Part print with two shaded views. Sizes in mm from the minimum x, y, z corner. A direction names the side the tool comes from. Round coordinates to 2 decimals unless told otherwise and drop trailing zeros. Order: outer loops, then holes, each group sorted by start corner. A loop starts at its lowest first (then second) coordinate and runs counter-clockwise, first axis right, second up. Notation, with made-up numbers: M 41,78 L 69,78 A8 cw 69,93 Z; hole C -34,54.5 d3. An arc over 180 degrees is marked long. Answer as a JSON object with one key per item and string values.
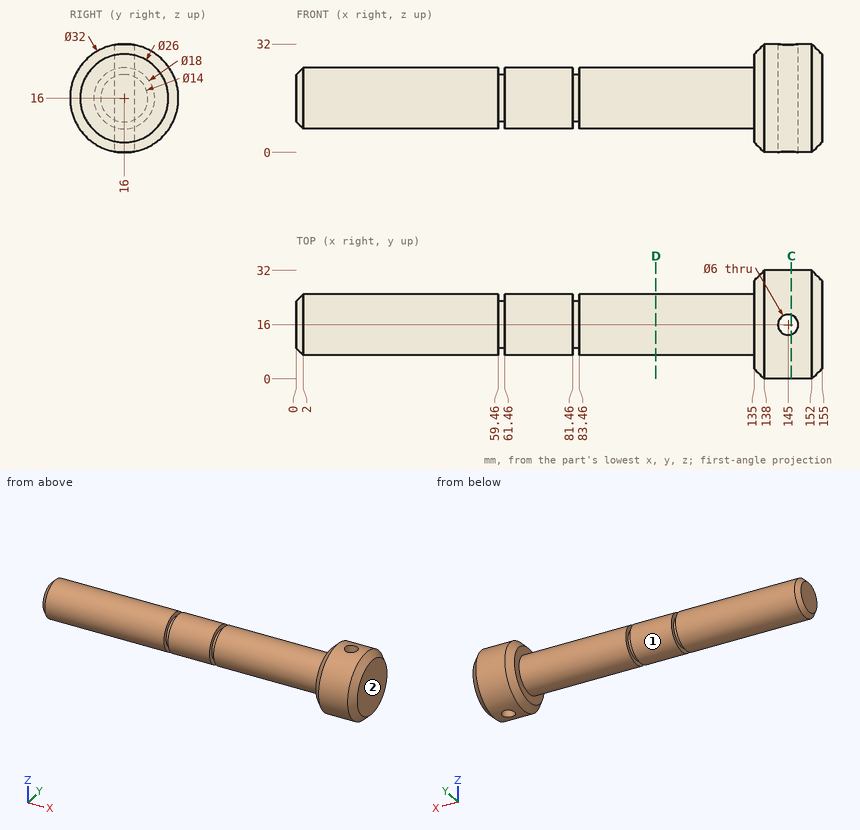
Item 1: Wall check: line 1 along Y through (x, z) = (145, 14); line 2 along X through (y, z) = (23.5, 9.5); line 3 along Y through (x, z) = (145, 7). Give the ranges that are in metal, low to high. Write a range as [from, to].
Worked answers:
{"line 1": "y = [0.13, 13], [19, 31.87]", "line 2": "x = [135, 155]", "line 3": "y = [2.77, 13], [19, 29.23]"}
Item 2: 3-axis set-ups, long thin cutter, end or side, ignore diameter. For the marked faces 1 and 2: which of +Z, -Z, +X, -X, +Y, -Y reach the whole face in a straight line?
Worked answers:
{"face 1": "-X", "face 2": "+Z, -Z, +X, +Y, -Y"}
Item 3: Drop flat-ended pins along their axis: pin 1 Ø12 at (x, z) = (29.5, 10.5) entering from -Y; pin 2 Ø3 at (x, y) = (50.5, 8) entering from +Z; pin 3 Ø1.5 at (x, y) = (46.5, 15.5) entering from +Z. Give the stop position or say it passes through.
Worked answers:
{"pin 1": "stops at y = 7", "pin 2": "stops at z = 22.22", "pin 3": "stops at z = 25"}
Item 4: Saw through at C-C on x = 146. List the corners of the cut face in (y, z).
Worked answers:
{"outline": "M 13.17,0.25 L 13.17,31.75 A16 ccw Z; M 18.83,0.25 A16 ccw 18.83,31.75 Z"}
Item 5: Saw through at D-D on x = 106. List the corners of the cut face in (y, z).
Worked answers:
{"outline": "C 16,16 d18"}
